Work out the finished part from the listing and answer in its coordinate system (mm). A direction names the side the tool comes from. Round coordinates to 2 decimals unless told otherwise and drop trailing zeros. Loops run counter-clockwise (first coordinate to the right, second up) from the corner with the lowest first, then second, coordinate; pieces in that order, holes last. Notation, with made-up numbers: (8.5, 45) - (42.5, 45) arc R16 ccw to (42.5, 72) - close; hole circle Ø2 at (75.5, 8). An arc over 180 degrees is marked (long way). Return JSON: item names as keys, results as strings.
from build123d import *

# Parameters (mm, degrees)
SKETCH1_R           = 95
SKETCH1_R_2         = 80
BOSS_EXTRUDE1_DEPTH = 50
CUT_EXTRUDE1_START  = -40
SKETCH2_R           = 80
CUT_EXTRUDE1_DEPTH  = 30


with BuildPart() as part:
    # Sketch1 → Boss-Extrude1 (new body)
    with BuildSketch(Plane.XY):
        with Locations((-599.884196758, -90)):
            Circle(SKETCH1_R)
        with Locations((-599.884196758, -90)):
            Circle(SKETCH1_R_2, mode=Mode.SUBTRACT)
    extrude(amount=BOSS_EXTRUDE1_DEPTH)

    # Sketch2 → Cut-Extrude1 (cut)
    with BuildSketch(Plane.XY.offset(50).offset(CUT_EXTRUDE1_START)):
        with BuildLine():
            ThreePointArc((-679.25673609, -100), (-673.794559359, -120.614674589), (-663.080125372, -139.05379299))
            Line((-663.080125372, -139.05379299), (-624.026332382, -100))
            Line((-624.026332382, -100), (-679.25673609, -100))
        make_face()
        with BuildLine():
            ThreePointArc((-694.356414897, -100), (-687.652752347, -126.354926075), (-673.757210649, -149.730878268))
            Line((-673.757210649, -149.730878268), (-663.080125372, -139.05379299))
            ThreePointArc((-663.080125372, -139.05379299), (-673.794559359, -120.614674589), (-679.25673609, -100))
            Line((-679.25673609, -100), (-694.356414897, -100))
        make_face()
        with BuildLine():
            Line((-609.884196758, -114.142135624), (-648.937989748, -153.195928613))
            ThreePointArc((-648.937989748, -153.195928613), (-630.498871347, -163.910362601), (-609.884196758, -169.372539332))
            Line((-609.884196758, -169.372539332), (-609.884196758, -114.142135624))
        make_face()
        with BuildLine():
            Line((-648.937989748, -153.195928613), (-659.615075026, -163.873013891))
            ThreePointArc((-659.615075026, -163.873013891), (-636.239122833, -177.768555589), (-609.884196758, -184.472218138))
            Line((-609.884196758, -184.472218138), (-609.884196758, -169.372539332))
            ThreePointArc((-609.884196758, -169.372539332), (-630.498871347, -163.910362601), (-648.937989748, -153.195928613))
        make_face()
        with BuildLine():
            Line((-589.884196758, -169.372539332), (-589.884196758, -184.472218138))
            ThreePointArc((-589.884196758, -184.472218138), (-563.529270683, -177.768555589), (-540.15331849, -163.873013891))
            Line((-540.15331849, -163.873013891), (-550.830403768, -153.195928613))
            ThreePointArc((-550.830403768, -153.195928613), (-569.269522169, -163.910362601), (-589.884196758, -169.372539332))
        make_face()
        with BuildLine():
            Line((-589.884196758, -114.142135624), (-589.884196758, -169.372539332))
            ThreePointArc((-589.884196758, -169.372539332), (-569.269522169, -163.910362601), (-550.830403768, -153.195928613))
            Line((-550.830403768, -153.195928613), (-589.884196758, -114.142135624))
        make_face()
        with BuildLine():
            Line((-575.742061134, -100), (-536.688268145, -139.05379299))
            ThreePointArc((-536.688268145, -139.05379299), (-525.973834157, -120.614674589), (-520.511657426, -100))
            Line((-520.511657426, -100), (-575.742061134, -100))
        make_face()
        with BuildLine():
            Line((-536.688268145, -139.05379299), (-526.011182867, -149.730878268))
            ThreePointArc((-526.011182867, -149.730878268), (-512.115641169, -126.354926075), (-505.41197862, -100))
            Line((-505.41197862, -100), (-520.511657426, -100))
            ThreePointArc((-520.511657426, -100), (-525.973834157, -120.614674589), (-536.688268145, -139.05379299))
        make_face()
        with BuildLine():
            Line((-536.688268145, -40.94620701), (-575.742061134, -80))
            Line((-575.742061134, -80), (-520.511657426, -80))
            ThreePointArc((-520.511657426, -80), (-525.973834157, -59.385325411), (-536.688268145, -40.94620701))
        make_face()
        with BuildLine():
            Line((-520.511657426, -80), (-505.41197862, -80))
            ThreePointArc((-505.41197862, -80), (-512.115641169, -53.645073925), (-526.011182867, -30.269121732))
            Line((-526.011182867, -30.269121732), (-536.688268145, -40.94620701))
            ThreePointArc((-536.688268145, -40.94620701), (-525.973834157, -59.385325411), (-520.511657426, -80))
        make_face()
        with BuildLine():
            Line((-589.884196758, -10.627460668), (-589.884196758, -65.857864376))
            Line((-589.884196758, -65.857864376), (-550.830403768, -26.804071387))
            ThreePointArc((-550.830403768, -26.804071387), (-569.269522169, -16.089637399), (-589.884196758, -10.627460668))
        make_face()
        with BuildLine():
            ThreePointArc((-540.15331849, -16.126986109), (-563.529270683, -2.231444411), (-589.884196758, 4.472218138))
            Line((-589.884196758, 4.472218138), (-589.884196758, -10.627460668))
            ThreePointArc((-589.884196758, -10.627460668), (-569.269522169, -16.089637399), (-550.830403768, -26.804071387))
            Line((-550.830403768, -26.804071387), (-540.15331849, -16.126986109))
        make_face()
        with BuildLine():
            ThreePointArc((-609.884196758, -10.627460668), (-630.498871347, -16.089637399), (-648.937989748, -26.804071387))
            Line((-648.937989748, -26.804071387), (-609.884196758, -65.857864376))
            Line((-609.884196758, -65.857864376), (-609.884196758, -10.627460668))
        make_face()
        with BuildLine():
            ThreePointArc((-609.884196758, 4.472218138), (-636.239122833, -2.231444411), (-659.615075026, -16.126986109))
            Line((-659.615075026, -16.126986109), (-648.937989748, -26.804071387))
            ThreePointArc((-648.937989748, -26.804071387), (-630.498871347, -16.089637399), (-609.884196758, -10.627460668))
            Line((-609.884196758, -10.627460668), (-609.884196758, 4.472218138))
        make_face()
        with BuildLine():
            ThreePointArc((-673.757210649, -30.269121732), (-687.652752347, -53.645073925), (-694.356414897, -80))
            Line((-694.356414897, -80), (-679.25673609, -80))
            ThreePointArc((-679.25673609, -80), (-673.794559359, -59.385325411), (-663.080125372, -40.94620701))
            Line((-663.080125372, -40.94620701), (-673.757210649, -30.269121732))
        make_face()
        with BuildLine():
            ThreePointArc((-663.080125372, -40.94620701), (-673.794559359, -59.385325411), (-679.25673609, -80))
            Line((-679.25673609, -80), (-624.026332382, -80))
            Line((-624.026332382, -80), (-663.080125372, -40.94620701))
        make_face()
        with Locations((-599.884196758, -90)):
            Circle(SKETCH2_R)
    extrude(amount=CUT_EXTRUDE1_DEPTH, mode=Mode.SUBTRACT)


solid = part.part
1) Flat-ended cylindrical pins translate along their axes: pin 1 (10 mm diameter, centred on x = -621.5, y = -160.5, fed in from -Z); pin 2 (4 mm diameter, centred on x = -652.5, z = 44, fed in from -Y); pin 3 (4.5 mm diameter, centred on y = -1, z = 30.5, fed in from -X); pin 4 (7.5 mm diameter, centred on y = 0.5, z = 17.5, fed in from +X). Find the tip coordinate at first contact, or state that the pin passes through.
Verdict:
{"pin 1": "passes through", "pin 2": "stops at y = -170.39", "pin 3": "stops at x = -609.88", "pin 4": "stops at x = -589.88"}
2) Section C-C (x = -631) is taken. Give the vertices of the cut face in (y, z).
Verdict:
{"outline": "(-179.76, 0) - (-163.7, 0) - (-163.7, 10) - (-179.76, 10) - close; (-179.76, 40) - (-163.7, 40) - (-163.7, 50) - (-179.76, 50) - close; (-16.3, 0) - (-0.24, 0) - (-0.24, 10) - (-16.3, 10) - close; (-16.3, 40) - (-0.24, 40) - (-0.24, 50) - (-16.3, 50) - close"}
3) Section D-D (x = -671) is taken. Give the vertices of the cut face in (y, z), and give its area (3 significant figures).
Verdict:
{"outline": "(-152.99, 0) - (-126.64, 0) - (-126.64, 10) - (-146.97, 10) - (-146.97, 40) - (-126.64, 40) - (-126.64, 50) - (-152.99, 50) - close; (-53.36, 0) - (-27.01, 0) - (-27.01, 50) - (-53.36, 50) - (-53.36, 40) - (-33.03, 40) - (-33.03, 10) - (-53.36, 10) - close", "area": "1,410 mm2"}
4) Find the intervals of material crossed by L1, parallel to Z at x = -587.5, y = -10.5; L2, parallel to X at y = -89, z = 44.5; L3, parallel to X at y = -170.5, z = 27, in increasing order.
Verdict:
{"L1": "z = 0 to 10, 40 to 50", "L2": "x = -694.88 to -679.88, -519.89 to -504.89", "L3": "x = -609.88 to -589.88"}
5) Section B-B (y = -90) is taken. Give the vertices of the cut face in (x, z), and give its area (3 significant figures).
Verdict:
{"outline": "(-694.88, 0) - (-679.88, 0) - (-679.88, 50) - (-694.88, 50) - close; (-519.88, 0) - (-504.88, 0) - (-504.88, 50) - (-519.88, 50) - close", "area": "1,500 mm2"}
6) Determine the mould class of faces 5 (the flat face through (-518, -125, 10)), 6 (the flat face through (-650, -153, 0)) for opening direction Z: pulls with the +Z half, pulls with the -Z half, needs draft (parallel to the pull), parting line crosses it, or undercut.
Verdict:
{"face 5": "undercut", "face 6": "pulls with the -Z half"}
7) A tool of negligible diameter and unlimited length cuts with its end or side. For faces 1 (the flat face through (-518, -125, 40)), 2 (the flat face through (-635, -172, 40)), 3 (the flat face through (-589.884, -177, 25)), 4 (the flat face through (-668.344, -35.682, 24.79)), from which of +Z, -Z, +X, -X, +Y, -Y can it reach the whole face along a straight path? Write none if from no direction.
Verdict:
{"face 1": "+X", "face 2": "-Y", "face 3": "+X, +Y, -Y", "face 4": "-X"}
8) Section A-A (z = 31) is taken. Count the separate pieces of the cut face and the enclosed holes in it, and give its area (3 significant figures).
Verdict:
{"separate pieces": "8", "enclosed holes": "0", "area": "2,410 mm2"}
